```python
from build123d import *

# Parameters (mm, degrees)
SKETCH1_R                               = 104.775
SKETCH1_R_2                             = 77.724
BOSS_EXTRUDE1_DEPTH                     = 0.381
F_9_16_0_5625_DIAMETER_HOLE1_AT_2_COUNT = 2
F_9_16_0_5625_DIAMETER_HOLE1_AT_2_PITCH = 141.053237967


with BuildPart() as part:
    # Sketch1 → Boss-Extrude1 (new body)
    with BuildSketch(Plane(origin=(0, 0, 0), x_dir=(1, 0, 0), z_dir=(0, 1, 0))):
        with Locations(Location((0, 0, 0), (0, 0, 90))):
            Circle(SKETCH1_R)
        with Locations(Location((0, 0, 0), (0, 0, 90))):
            Circle(SKETCH1_R_2, mode=Mode.SUBTRACT)
    extrude(amount=BOSS_EXTRUDE1_DEPTH)

    # Sketch2 → 9/16 (0.5625) Diameter Hole1 (revolve, cut)
    with BuildSketch(Plane(origin=(-62.8586, 0.381, -62.865), x_dir=(0, 0, 1), z_dir=(1, 0, 0))):
        Polygon((0, 0), (0, 20.172398047), (7.14375, 15.88), (7.14375, 0), align=None)
    f_9_16_0_5625_diameter_hole1 = revolve(axis=Axis((-62.8586, 6.731, -62.865), (0, -1, 0)), mode=Mode.SUBTRACT)

    # 9/16 (0.5625) Diameter Hole1 at 2: 9/16 (0.5625) Diameter Hole1 ×2
    with Locations(*[Vector(0.9914412601618559, 0, 0.1305535432252662) * (i * F_9_16_0_5625_DIAMETER_HOLE1_AT_2_PITCH) for i in range(1, F_9_16_0_5625_DIAMETER_HOLE1_AT_2_COUNT)]):
        add(f_9_16_0_5625_diameter_hole1, mode=Mode.SUBTRACT)

    # Mirror1: 9/16 (0.5625) Diameter Hole1 across plane
    add(f_9_16_0_5625_diameter_hole1.mirror(Plane.XY), mode=Mode.SUBTRACT)

    # Mirror1 copy 1 sketch → Mirror1 copy 1 (revolve, cut)
    with BuildSketch(Plane(origin=(76.9874, 0.381, 44.45), x_dir=(0, 0, -1), z_dir=(1, 0, 0))):
        Polygon((0, 0), (0, -20.172398047), (7.14375, -15.88), (7.14375, 0), align=None)
    revolve(axis=Axis((76.9874, 6.731, 44.45), (0, 1, 0)), mode=Mode.SUBTRACT)


solid = part.part
```
Can you work these out from the model? Positions are in its coordinate system, mm. Coordinates: 2 decimals unless noted, no trailing zeros. Loops run counter-clockwise (first coordinate to the right, second up) from the corner with the lowest first, then second, coordinate; pieces in that order, holes last. Notation, with made-up numbers: (28.5, 36) -> (60.5, 36) arc R28 cw to (60.5, 64) -> close; hole circle Ø2 at (-19, 81). An arc over 180 degrees is marked (long way). Answer as a JSON object with one key per item and string values.
1) Imagine slicing it at C-C (z = -63). Please give me the cut outline in (x, y).
Results:
{"outline": "(-83.72, 0) -> (-70, 0) -> (-70, 0.38) -> (-83.72, 0.38) -> close; (-55.72, 0) -> (-45.52, 0) -> (-45.52, 0.38) -> (-55.72, 0.38) -> close; (45.52, 0) -> (83.72, 0) -> (83.72, 0.38) -> (45.52, 0.38) -> close"}
2) Imagine slicing it at A-A (x = 0). Please give me the cut outline in (y, z) (3 decimals).
Results:
{"outline": "(0, -104.775) -> (0.381, -104.775) -> (0.381, -77.724) -> (0, -77.724) -> close; (0, 77.724) -> (0.381, 77.724) -> (0.381, 104.775) -> (0, 104.775) -> close"}
3) Thinking about a two-plate mould opening in X: for faces 1 (the face through (102.283, 0.188, 22.713)), 2 (the face through (70.964, 0.193, 40.61)), 3 (the face through (-8, 0.381, 78)), which applies, pulls with the +X half, pulls with the -X half, needs draft (parallel to the pull), parting line crosses it, or undercut?
Results:
{"face 1": "parting line crosses it", "face 2": "undercut", "face 3": "needs draft"}
4) If I drill on line 1 (Z direction, x = -0.5, y = 0.1); line 2 (X direction, y = 0.1, z = -44.45); line 3 (X direction, y = 0.2, z = 41.5), over which ranges is the centre line in solid material (lowest first)?
Results:
{"line 1": "z = -104.77 to -77.72, 77.72 to 104.77", "line 2": "x = -94.88 to -63.76, 63.76 to 69.84, 84.13 to 94.88", "line 3": "x = -96.21 to -65.72, 65.72 to 70.48, 83.49 to 96.21"}
5) Imagine slicing it at D-D (y = 0.3). Count the separate pieces of the cut face and the enclosed holes in it, then the cut area to 3 significant figures.
Results:
{"separate pieces": "1", "enclosed holes": "5", "area": "14,900 mm^2"}
6) Imagine slicing it at B-B (z = 0). Please give me the cut outline in (x, y) (3 decimals), then the cut area to 3 significant figures.
Results:
{"outline": "(-104.775, 0) -> (-77.724, 0) -> (-77.724, 0.381) -> (-104.775, 0.381) -> close; (77.724, 0) -> (104.775, 0) -> (104.775, 0.381) -> (77.724, 0.381) -> close", "area": "20.6 mm^2"}
7) For P1, Ø8.5, axis at x = 76.99, z = 44.45, coming from the -Y side; P2, Ø16.5, axis at x = -62.86, z = 62.86, coming from the +Y side, each with a flat end and sliding along its axis, tell me the tip position at first contact or that it passes through.
Results:
{"P1": "passes through", "P2": "stops at y = 0.38"}
